from build123d import *

# Parameters (mm, degrees)
SKETCH1_R             = 5
BOSS_EXTRUDE1_DEPTH   = 321
M6_TAPPED_HOLE1_D     = 5
M6_TAPPED_HOLE1_DEPTH = 15
M6_TAPPED_HOLE1_TIP   = 1.502151548
M6_TAPPED_HOLE2_D     = 5
M6_TAPPED_HOLE2_DEPTH = 15
M6_TAPPED_HOLE2_TIP   = 1.502151548


with BuildPart() as part:
    # Sketch1 → Boss-Extrude1 (new body)
    with BuildSketch(Plane.XY):
        Circle(SKETCH1_R)
    extrude(amount=BOSS_EXTRUDE1_DEPTH)

    # M6 Tapped Hole1
    with Locations(Plane.XY.offset(321)):
        with Locations((0, 0)):
            Hole(M6_TAPPED_HOLE1_D / 2, depth=M6_TAPPED_HOLE1_DEPTH)
            with Locations((0, 0, -(M6_TAPPED_HOLE1_DEPTH + M6_TAPPED_HOLE1_TIP / 2))):  # 118° drill point
                Cone(0, M6_TAPPED_HOLE1_D / 2, M6_TAPPED_HOLE1_TIP, mode=Mode.SUBTRACT)

    # M6 Tapped Hole2
    with Locations(Plane(origin=(0, 0, 0), x_dir=(-1, 0, 0), z_dir=(0, 0, -1))):
        with Locations((0, 0)):
            Hole(M6_TAPPED_HOLE2_D / 2, depth=M6_TAPPED_HOLE2_DEPTH)
            with Locations((0, 0, -(M6_TAPPED_HOLE2_DEPTH + M6_TAPPED_HOLE2_TIP / 2))):  # 118° drill point
                Cone(0, M6_TAPPED_HOLE2_D / 2, M6_TAPPED_HOLE2_TIP, mode=Mode.SUBTRACT)


solid = part.part
Check sheet for the modelled part. Datum: model origin and axes. Units: mm. A direction names the side the tool comes from. Round coordinates to 2 decimals unless told otherwise and drop trailing zeros. Write each loop counter-clockwise with the first axis right and the second up, starting at its lowest first coordinate (ties: lowest second). Pieces come first, ordered by that corner, then holes. Notation, with made-up numbers: (-36, 26) -> (-9, 26) arc R26 cw to (-9, 54) -> close; hole circle Ø3 at (-33, 69.25). An arc over 180 degrees is marked (long way). Answer as CSV lines item,"result". Start each with the question number.
1) Go/stop test with flat-tipped pins: P1, Ø1.5, axis at y = 3.5, z = 253.5, coming from the +X side; P2, Ø6, axis at y = -4, z = 141.5, coming from the -X side; P3, Ø1, axis at y = -2, z = 59.5, coming from the +X side. Record where each tip stops, or that it passes through.
2) Tool access check on faces 1 (the cylindrical face through (-0.54, -2.44, 7.6)), 2 (the flat face through (2, -2, 321)). Record the directions out of +Z, -Z, +X, -X, +Y, -Y that give a thin tool (end or side, any length) a straight path to the whole face; none if there is none.
3) Release check for a two-part mould opening along X. For faces 3 (the flat face through (2, -2, 0)), 4 (the cylindrical face through (-1.08, -4.88, 158.25)), 5 (the cylindrical face through (0.54, -2.44, 313.4)) record: pulls with the +X half, pulls with the -X half, needs draft (parallel to the pull), parting line crosses it, or undercut.
4) Section check A-A on z = 207. Enter the section's corners in (x, y).
5) Material ranges on line 1 (Y direction, x = 0, z = 11); line 2 (X direction, y = -0.5, z = 160.5); line 3 (Y direction, x = 1.75, z = 30.5), recorded low to high. Write a range as from..to.
Found:
1,P1,"stops at x = 4.18"
1,P2,"stops at x = -4.9"
1,P3,"stops at x = 4.77"
2,face 1,"-Z"
2,face 2,"+Z, +X, -X, +Y, -Y"
3,face 3,"needs draft"
3,face 4,"parting line crosses it"
3,face 5,"undercut"
4,outline,"circle Ø10 at (0, 0)"
5,line 1,"y = -5..-2.5, 2.5..5"
5,line 2,"x = -4.97..4.97"
5,line 3,"y = -4.68..4.68"
